Work out the finished part from the listing and answer in its coordinate system (mm). A direction names the side the tool comes from. Round coordinates to 2 decimals unless told otherwise and drop trailing zeros. Order: outer loops, then holes, each group sorted by start corner. A loop starts at its lowest first (then second) coordinate and runs counter-clockwise, first axis right, second up. Notation, with made-up numbers: (6.25, 10.5) - (18.25, 10.5) arc R20 cw to (18.25, 29.5) - close; hole circle Ø2 at (55.25, 0.25). An arc over 180 degrees is marked (long way). Use one line per item in the form item = value. Start each with the question number.
Q1. For a pull along Y with two mould halves and no side action, classify faces 6 (the cylindrical face through (-81.414, -8.872, 0.658)), 7 (the flat face through (-233, 0, -55)), 8 (the flat face through (-8, -25, -1)) as +Y half, -Y half, draft (parallel to the pull), parting line (faces both ways), or undercut.
Q2. Find the intervals of material crossed by line 1 (Y direction, x = -76.8, z = 39); line 2 (Y direction, x = -235, z = 40); line 3 (X direction, y = 4, z = -39), in increasing order. Write a range as [from, to].
Q3. Given P1, Ø12, axis at y = -10.5, z = 70.5, coming from the -X side; P2, Ø16, axis at x = 244, y = 0, coming from the -Z side; P3, Ø13, axis at x = -97.5, y = 1, coming from the -Z side, each flat-ended and moving along its own axis, determine where each tip first touches the part or whether it passes through.
Q4. The part is cut by section A-A on z = 7.5. Determine the outline of the cut face in (x, y), plus the area to 3 significant figures.
Q5. The part is cut by section B-B on x = -145.5. Determine the outline of the cut face in (y, z), plus the area to 3 significant figures.
Q6. Which of the six approach directions +Z, -Z, +X, -X, +Y, -Y give full straight-line access (tool end or side, diameter ignored) to faces 1 (the flat face through (234, 0, 130)), 2 (the cylindrical face through (-71.705, 0.224, 35.17)), 3 (the flat face through (3, -22, 1)), 4 (the flat face through (-8, 25, -1)), 5 (the cylindrical face through (252.346, 2.628, -105.918))?
from build123d import *

# Parameters (mm, degrees)
SKETCH_1_W                    = 466
SKETCH_1_H                    = 110
EXTRUDE_1_DEPTH               = 50
SKETCH_2_W                    = 456
SKETCH_2_H                    = 5
CUT_EXTRUDE_1_DEPTH           = 250.337121183
SKETCH_3_W                    = 456
SKETCH_3_H                    = 5
CUT_EXTRUDE_2_DEPTH           = 250.337121183
SKETCH_4_W                    = 94
SKETCH_4_H                    = 44
CUT_EXTRUDE_3_DEPTH           = 456
SKETCH_5_W                    = 10
SKETCH_5_H                    = 94
SKETCH_6_W                    = 25
SKETCH_6_H                    = 260
HOLE_WIZARD_8_5_8_5_1_D       = 8.5
HOLE_WIZARD_8_5_8_5_1_DEPTH   = 10
HOLE_WIZARD_M12_3_D           = 10.2
HOLE_WIZARD_M12_3_DEPTH       = 29.25
HOLE_WIZARD_M12_3_TIP         = 3.064389157
HOLE_WIZARD_M12_4_D           = 10.2
HOLE_WIZARD_M12_4_DEPTH       = 29.25
HOLE_WIZARD_M12_4_TIP         = 3.064389157
HOLE_WIZARD_10_2_10_2_2_D     = 10.2
HOLE_WIZARD_10_2_10_2_2_DEPTH = 29.25
HOLE_WIZARD_10_2_10_2_2_TIP   = 3.064389157
CHAMFER_1_SIZE                = 1
FILLET_1_R                    = 3
CHAMFER_2_SIZE                = 5
HOLE_WIZARD_M20_1_D           = 17.5
HOLE_WIZARD_M20_1_DEPTH       = 47.5
HOLE_WIZARD_M20_1_TIP         = 5.257530416
HOLE_WIZARD_M20_2_D           = 17.5
HOLE_WIZARD_M20_2_DEPTH       = 47.5
HOLE_WIZARD_M20_2_TIP         = 5.257530416


with BuildPart() as part:
    # 草图1 → 凸台-拉伸1 (new body)
    with BuildSketch(Plane(origin=(0, 25, 0), x_dir=(1, 0, 0), z_dir=(0, 1, 0))):
        with Locations((-5, 0)):
            Rectangle(SKETCH_1_W, SKETCH_1_H)
    extrude(amount=-EXTRUDE_1_DEPTH)

    # 草图2 → 切除-拉伸1 (cut, through all)
    with BuildSketch(Plane.XZ.offset(25)):
        with Locations((0, -52.5)):
            Rectangle(SKETCH_2_W, SKETCH_2_H)
    extrude(amount=-CUT_EXTRUDE_1_DEPTH, mode=Mode.SUBTRACT)

    # 草图3 → 切除-拉伸2 (cut, through all)
    with BuildSketch(Plane.XZ.offset(25)):
        with Locations((0, 52.5)):
            Rectangle(SKETCH_3_W, SKETCH_3_H)
    extrude(amount=-CUT_EXTRUDE_2_DEPTH, mode=Mode.SUBTRACT)

    # 草图4 → 切除-拉伸3 (cut)
    with BuildSketch(Plane(origin=(228, 0, 0), x_dir=(0, 0, -1), z_dir=(1, 0, 0))):
        Rectangle(SKETCH_4_W, SKETCH_4_H)
    extrude(amount=-CUT_EXTRUDE_3_DEPTH, mode=Mode.SUBTRACT)

    # 草图5 → 旋转1 (revolve)
    with BuildSketch(Plane.XZ, mode=Mode.PRIVATE) as revolve_1_sk:
        with Locations((-71.8, 0)):
            Rectangle(SKETCH_5_W, SKETCH_5_H)
    revolve(revolve_1_sk.sketch.rotate(Axis((-76.8, 0, 47), (0, 0, -1)), 180), axis=Axis((-76.8, 0, 47), (0, 0, -1)))

    # 草图6 → 旋转2 (revolve)
    with BuildSketch(Plane(origin=(0, 0, 0), x_dir=(1, 0, 0), z_dir=(0, 1, 0))):
        with Locations((231.5, 0)):
            Rectangle(SKETCH_6_W, SKETCH_6_H)
    revolve(axis=Axis((244, 0, 130), (0, 0, -1)))

    # Ø8.5 (8.5) 直径孔1
    with Locations(Plane(origin=(-228, 0, 0), x_dir=(0, 0, -1), z_dir=(1, 0, 0))):
        with Locations((40, 10), (-40, 10)):
            Hole(HOLE_WIZARD_8_5_8_5_1_D / 2, depth=HOLE_WIZARD_8_5_8_5_1_DEPTH)

    # M12 螺纹孔3
    with Locations(Plane.XY.offset(50)):
        with Locations((-76.8, 0)):
            Hole(HOLE_WIZARD_M12_3_D / 2, depth=HOLE_WIZARD_M12_3_DEPTH)
            with Locations((0, 0, -(HOLE_WIZARD_M12_3_DEPTH + HOLE_WIZARD_M12_3_TIP / 2))):  # 118° drill point
                Cone(0, HOLE_WIZARD_M12_3_D / 2, HOLE_WIZARD_M12_3_TIP, mode=Mode.SUBTRACT)

    # M12 螺纹孔4
    with Locations(Plane(origin=(0, 0, -50), x_dir=(-1, 0, 0), z_dir=(0, 0, -1))):
        with Locations((76.8, 0)):
            Hole(HOLE_WIZARD_M12_4_D / 2, depth=HOLE_WIZARD_M12_4_DEPTH)
            with Locations((0, 0, -(HOLE_WIZARD_M12_4_DEPTH + HOLE_WIZARD_M12_4_TIP / 2))):  # 118° drill point
                Cone(0, HOLE_WIZARD_M12_4_D / 2, HOLE_WIZARD_M12_4_TIP, mode=Mode.SUBTRACT)

    # Ø10.2 (10.2) 直径孔2
    with Locations(Plane(origin=(0, 0, -50), x_dir=(-1, 0, 0), z_dir=(0, 0, -1))):
        with Locations((76.8, 0)):
            Hole(HOLE_WIZARD_10_2_10_2_2_D / 2, depth=HOLE_WIZARD_10_2_10_2_2_DEPTH)
            with Locations((0, 0, -(HOLE_WIZARD_10_2_10_2_2_DEPTH + HOLE_WIZARD_10_2_10_2_2_TIP / 2))):  # 118° drill point
                Cone(0, HOLE_WIZARD_10_2_10_2_2_D / 2, HOLE_WIZARD_10_2_10_2_2_TIP, mode=Mode.SUBTRACT)

    # 倒角1
    chamfer_1_edges = [part.edges().sort_by_distance(p)[0] for p in [
        (269, 0, 130),
        (269, 0, -130),
    ]]
    chamfer(chamfer_1_edges, length=CHAMFER_1_SIZE)

    # 圆角1
    fillet_1_edges = [part.edges().sort_by_distance(p)[0] for p in [
        (0, 25, -50),
        (0, -25, -50),
        (0, 25, 50),
        (0, -25, 50),
    ]]
    fillet(fillet_1_edges, radius=FILLET_1_R)

    # 倒角2
    chamfer_2_edges = [part.edges().sort_by_distance(p)[0] for p in [
        (-233, 25, -55),
        (-233, -25, -55),
        (-233, -25, 55),
        (-233, 25, 55),
    ]]
    chamfer(chamfer_2_edges, length=CHAMFER_2_SIZE)

    # M20 螺纹孔1
    with Locations(Plane.XY.offset(130)):
        with Locations((244, 0)):
            Hole(HOLE_WIZARD_M20_1_D / 2, depth=HOLE_WIZARD_M20_1_DEPTH)
            with Locations((0, 0, -(HOLE_WIZARD_M20_1_DEPTH + HOLE_WIZARD_M20_1_TIP / 2))):  # 118° drill point
                Cone(0, HOLE_WIZARD_M20_1_D / 2, HOLE_WIZARD_M20_1_TIP, mode=Mode.SUBTRACT)

    # M20 螺纹孔2
    with Locations(Plane(origin=(0, 0, -130), x_dir=(-1, 0, 0), z_dir=(0, 0, -1))):
        with Locations((-244, 0)):
            Hole(HOLE_WIZARD_M20_2_D / 2, depth=HOLE_WIZARD_M20_2_DEPTH)
            with Locations((0, 0, -(HOLE_WIZARD_M20_2_DEPTH + HOLE_WIZARD_M20_2_TIP / 2))):  # 118° drill point
                Cone(0, HOLE_WIZARD_M20_2_D / 2, HOLE_WIZARD_M20_2_TIP, mode=Mode.SUBTRACT)


solid = part.part
Found:
q1.face_6 = undercut
q1.face_7 = draft
q1.face_8 = -Y half
q2.line_1 = [-25, -22], [-10, -5.1], [5.1, 10], [22, 25]
q2.line_2 = [-25, 5.75], [14.25, 25]
q2.line_3 = [-238, -228], [-85.97, -79.96], [-73.64, -67.63], [219.32, 268.68]
q3.P1 = 219.41
q3.P2 = -82.05
q3.P3 = -50
q4.outline = (-238, -25) - (228, -25) - (228, -22) - (-228, -22) - (-228, 22) - (228, 22) - (228, 25) - (-238, 25) - close; circle Ø20 at (-76.8, 0); circle Ø50 at (244, 0)
q4.area = 5,510 mm²
q5.outline = (-25, -47) arc R3 ccw to (-22, -50) - (22, -50) arc R3 ccw to (25, -47) - (25, 47) arc R3 ccw to (22, 50) - (-22, 50) arc R3 ccw to (-25, 47) - close; hole (-22, -47) - (22, -47) - (22, 47) - (-22, 47) - close
q5.area = 856 mm²
q6.face_1 = +Z, +X, -X, +Y, -Y
q6.face_2 = +Z
q6.face_3 = none
q6.face_4 = +Z, -Z, +X, -X, +Y
q6.face_5 = -Z
